```python
from build123d import *

# Parameters (mm, degrees)
SKETCH1_R           = 6.5
SKETCH1_R_2         = 3
BOSS_EXTRUDE1_DEPTH = 4.5
CHAMFER1_SIZE       = 0.5


with BuildPart() as part:
    # Sketch1 → Boss-Extrude1 (new body)
    with BuildSketch(Plane(origin=(0, 0, 0), x_dir=(1, 0, 0), z_dir=(0, 1, 0))):
        with Locations(Location((0, 0, 0), (0, 0, 270))):
            Circle(SKETCH1_R)
        with Locations(Location((0, 0, 0), (0, 0, 270))):
            Circle(SKETCH1_R_2, mode=Mode.SUBTRACT)
    extrude(amount=BOSS_EXTRUDE1_DEPTH)

    # Chamfer1
    chamfer1_edges = [part.edges().sort_by_distance(p)[0] for p in [
        (0, 0, -6.5),
        (0, 4.5, -6.5),
        (0, 0, -3),
        (0, 4.5, -3),
    ]]
    chamfer(chamfer1_edges, length=CHAMFER1_SIZE)


solid = part.part
```
The listing builds one solid part. Answer for the finished solid, in the listing's coordinates (mm). Coordinates: 2 decimals unless noted, no trailing zeros. Write each loop counter-clockwise with the first axis right and the second up, starting at its lowest first coordinate (ties: lowest second). Pieces come first, ordered by that corner, then holes. Notation, with made-up numbers: M 49.25,73 L 75.25,73 A33 ccw 75.25,108 Z; hole C 68.25,-24.5 d11. An arc over 180 degrees is marked long. Use a Markdown table: item, result. Add a question column.
1. Given P1, Ø5.5, axis at x = 0, z = 0, coming from the -Y side; P2, Ø2, axis at x = -4.5, y = 4, coming from the -Z side, each flat-ended and moving along its own axis, determine where each tip first touches the part or whether it passes through.
2. Section B-B (x = 0) is taken. Give the vertices of the cut face in (y, z).
3. Section A-A (z = 0) is taken. Give the vertices of the cut face in (x, y), plus the area to 3 significant figures.
4. Section C-C (y = 2.6) is taken. Give the vertices of the cut face in (x, z), plus the area to 3 significant figures.
5. For a pull along Z with two mould halves and no side action, classify faces 1 (the flat face through (-3, 0, 3)), 2 (the cylindrical face through (0.9, 2.23, 2.86)), 3 (the cylindrical face through (-3.955, 2.226, -5.158)) as +Z half, -Z half, draft (parallel to the pull), parting line (faces both ways), or undercut.
6. Straight lines are drawn through the part: line 1 along X through (y, z) = (3.1, -0.25); line 2 along X through (y, z) = (2.3, 0.75); line 3 along Z through (x, y) = (-0.5, 1.65). For each, find the intervals that lie inside material, in ascending order. Write a range as [from, to].
Data:
| question | item | result |
|---|---|---|
| 1 | P1 | passes through |
| 1 | P2 | stops at z = -5.48 |
| 2 | outline | M 0,-6 L 0.5,-6.5 L 4,-6.5 L 4.5,-6 L 4.5,-3.5 L 4,-3 L 0.5,-3 L 0,-3.5 Z; M 0,3.5 L 0.5,3 L 4,3 L 4.5,3.5 L 4.5,6 L 4,6.5 L 0.5,6.5 L 0,6 Z |
| 3 | outline | M -6.5,0.5 L -6,0 L -3.5,0 L -3,0.5 L -3,4 L -3.5,4.5 L -6,4.5 L -6.5,4 Z; M 3,0.5 L 3.5,0 L 6,0 L 6.5,0.5 L 6.5,4 L 6,4.5 L 3.5,4.5 L 3,4 Z |
| 3 | area | 30.5 mm2 |
| 4 | outline | C 0,0 d13; hole C 0,0 d6 |
| 4 | area | 104 mm2 |
| 5 | face 1 | draft |
| 5 | face 2 | undercut |
| 5 | face 3 | parting line |
| 6 | line 1 | x = [-6.5, -2.99], [2.99, 6.5] |
| 6 | line 2 | x = [-6.46, -2.9], [2.9, 6.46] |
| 6 | line 3 | z = [-6.48, -2.96], [2.96, 6.48] |
